```python
from build123d import *

# Parameters (mm, degrees)
BOSS_EXTRUDE1_DEPTH      = 150
BOSS_EXTRUDE1_DEPTH_BACK = 270
SKETCH1_R                = 35
SKETCH2_R                = 50
BOSS_EXTRUDE2_DEPTH      = 60
CHAMFER1_SIZE            = 4
CUT_EXTRUDE1_DEPTH       = 10


with BuildPart() as part:
    # Sketch1 → Boss-Extrude1 (new, two sides: drawn at the far end of the back side and taken through both)
    with BuildSketch(Plane.XY.offset(-BOSS_EXTRUDE1_DEPTH_BACK)):
        Circle(SKETCH1_R)
    extrude(amount=BOSS_EXTRUDE1_DEPTH + BOSS_EXTRUDE1_DEPTH_BACK)

    # Sketch2 → Boss-Extrude2 (add, symmetric)
    with BuildSketch(Plane.XY):
        Circle(SKETCH2_R)
    extrude(amount=BOSS_EXTRUDE2_DEPTH, both=True)

    # Chamfer1
    chamfer1_edges = [part.edges().sort_by_distance(p)[0] for p in [
        (-35, 0, -270),
        (-35, 0, 150),
        (-50, 0, -60),
        (-50, 0, 60),
    ]]
    chamfer(chamfer1_edges, length=CHAMFER1_SIZE)

    # Sketch3 → Cut-Extrude1 (cut)
    with BuildSketch(Plane(origin=(0, 35, 0), x_dir=(1, 0, 0), z_dir=(0, 1, 0))):
        with BuildLine():
            Line((-7.5, 305), (7.5, 305))
            Line((7.5, 305), (7.5, 235))
            ThreePointArc((7.5, 235), (0, 227.5), (-7.5, 235))
            Line((-7.5, 235), (-7.5, 305))
        make_face()
    extrude(amount=-CUT_EXTRUDE1_DEPTH, mode=Mode.SUBTRACT)


solid = part.part
```
Input: part model. Units: mm. Frame: model coordinates. A direction names the side the tool comes from. Round coordinates to 2 decimals unless told otherwise and drop trailing zeros. Loops run counter-clockwise (first coordinate to the right, second up) from the corner with the lowest first, then second, coordinate; pieces in that order, holes last. Notation, with made-up numbers: (60.5, 56) -> (70.5, 56) arc R9 ccw to (70.5, 63) -> close; hole circle Ø6 at (-10, 55.5). An arc over 180 degrees is marked (long way). One line per item, written item: value.
(1) Section C-C (z = -42.5). Return the cut outline in (x, y), plus the area to 3 significant figures.
Geometry check:
outline: circle Ø100 at (0, 0)
area: 7,850 mm2
(2) Section B-B (y = 0). Return the cut outline in (x, z), plus the area to 3 significant figures.
Geometry check:
outline: (-50, -56) -> (-46, -60) -> (-35, -60) -> (-35, -266) -> (-31, -270) -> (31, -270) -> (35, -266) -> (35, -60) -> (46, -60) -> (50, -56) -> (50, 56) -> (46, 60) -> (35, 60) -> (35, 146) -> (31, 150) -> (-31, 150) -> (-35, 146) -> (-35, 60) -> (-46, 60) -> (-50, 56) -> close
area: 32,900 mm2
(3) Section D-D (z = -195.5). Return the cut outline in (x, y).
Geometry check:
outline: circle Ø70 at (0, 0)
(4) Pin query (flat end, axial travel): pin 1 (4 mm diameter, centred on x = 4, z = -27, fed in from -Y); pin 2 (1.5 mm diameter, centred on x = 30.5, z = 88.5, fed in from +Y); pin 3 (7.5 mm diameter, centred on y = 31.5, z = -250.5, fed in from +X). Return the tip coordinate at first contact, or that it passes through.
Geometry check:
pin 1: y = -49.96
pin 2: y = 18.44
pin 3: x = 21.33
(5) Section A-A (x = 0). Return the cut outline in (y, z).
Geometry check:
outline: (-50, -56) -> (-46, -60) -> (-35, -60) -> (-35, -266) -> (-31, -270) -> (25, -270) -> (25, -227.5) -> (35, -227.5) -> (35, -60) -> (46, -60) -> (50, -56) -> (50, 56) -> (46, 60) -> (35, 60) -> (35, 146) -> (31, 150) -> (-31, 150) -> (-35, 146) -> (-35, 60) -> (-46, 60) -> (-50, 56) -> close
(6) Mould query, pull axis X, two halves, no side actions, for faces 1 (the face through (-7.5, 30, -252)), 2 (the face through (0.16, 30.07, -227.5)), 3 (the face through (-24.75, -18.98, 149.81)), 4 (the face through (0, 0, 150)). Classes: pulls with the +X half, pulls with the -X half, needs draft (parallel to the pull), parting line crosses it, or undercut.
Geometry check:
face 1: undercut
face 2: undercut
face 3: parting line crosses it
face 4: needs draft
(7) Material intervals for line 1 (Z direction, x = 13.5, y = 38); line 2 (Y direction, x = 1.5, z = 42); line 3 (X direction, y = 1, z = -110), sorted ascending. Write a range as [from, to].
Geometry check:
line 1: [-60, 60]
line 2: [-49.98, 49.98]
line 3: [-34.99, 34.99]
(8) Set-up query: faces 5 (the face through (0, 0, -270)), 6 (the face through (47.69, 15.02, 0.78)), 7 (the face through (7.5, 30, -253)), 8 (the face through (-17, 31, -60)), 9 (the face through (-17, 31, 60)). Return all of +Z, -Z, +X, -X, +Y, -Y with unobstructed straight access to the full face (end or side cutting, diameter ignored); none if empty.
Geometry check:
face 5: -Z, +X, -X, +Y, -Y
face 6: +Z, -Z
face 7: -Z, +Y
face 8: -Z
face 9: +Z
